Design review of the part built by this model. Coordinates are the model's own, in mm. Coordinates: 2 decimals unless noted, no trailing zeros. Loops run counter-clockwise (first coordinate to the right, second up) from the corner with the lowest first, then second, coordinate; pieces in that order, holes last. Notation, with made-up numbers: M -26.5,55 L -16.5,55 A36 ccw -16.5,92 Z; hole C 63.25,29 d1. An arc over 180 degrees is marked long. Answer as a JSON object with one key per item and string values. Group by question number.
1. Consider section A-A (x = 130). State the section outline as (y, z) points.
2. To check wall thickness, follow probe 1 along Y at (x, z) = (130, 5.75); probe 2 along Y at (x, z) = (56, 7); probe 3 along X at (y, z) = (6.5, 7.5). State the ranges of each line that lie inside material, in increasing order.
3. Consider section B-B (z = 6). State the section outline as (x, y) points, then the cut area to 3 significant figures.
4. Draft analysis for pull direction X (two halves, no side actions). For faces 1 (the flat face through (170, 35, 4)), 2 (the flat face through (0, 35, 4)), 3 (the cylindrical face through (49.154, 36.445, 4.056)), 4 (the cylindrical face through (123.506, 30.286, 4.056)), state which applies: +X half, -X half, draft (parallel to the pull), parting line (faces both ways), or undercut.
5. Consider section C-C (y = 30). State the section outline as (x, z) points.
from build123d import *

# Parameters (mm, degrees)
EXTRUDE_1_DEPTH     = 8
SKETCH_2_R          = 6.5
CUT_EXTRUDE_1_DEPTH = 8


with BuildPart() as part:
    # 草图1 → 凸台-拉伸1 (new body)
    with BuildSketch(Plane.XY):
        Polygon((10, 0), (160, 0), (170, 10), (170, 60), (0, 60), (0, 10), align=None)
    extrude(amount=EXTRUDE_1_DEPTH)

    # 草图2 → 切除-拉伸1 (cut)
    with BuildSketch(Plane.XY.offset(8)):
        with Locations((50, 30)):
            Circle(SKETCH_2_R)
        with Locations((130, 30)):
            Circle(SKETCH_2_R)
    extrude(amount=-CUT_EXTRUDE_1_DEPTH, mode=Mode.SUBTRACT)


solid = part.part
Findings below:
{
 "1": {"outline": "M 0,0 L 23.5,0 L 23.5,8 L 0,8 Z; M 36.5,0 L 60,0 L 60,8 L 36.5,8 Z"},
 "2": {"probe 1": "y = 0 to 23.5, 36.5 to 60", "probe 2": "y = 0 to 27.5, 32.5 to 60", "probe 3": "x = 3.5 to 166.5"},
 "3": {"outline": "M 0,10 L 10,0 L 160,0 L 170,10 L 170,60 L 0,60 Z; hole C 50,30 d13; hole C 130,30 d13", "area": "9,830 mm^2"},
 "4": {"face 1": "+X half", "face 2": "-X half", "face 3": "undercut", "face 4": "undercut"},
 "5": {"outline": "M 0,0 L 43.5,0 L 43.5,8 L 0,8 Z; M 56.5,0 L 123.5,0 L 123.5,8 L 56.5,8 Z; M 136.5,0 L 170,0 L 170,8 L 136.5,8 Z"}
}
